Model file for the job. Use its own axes, mm. Face numbers are marked on the shaded views. A direction names the side the tool comes from. Round coordinates to 2 decimals unless told otherwise and drop trailing zeros. Loops run counter-clockwise (first coordinate to the right, second up) from the corner with the lowest first, then second, coordinate; pieces in that order, holes last. Notation, with made-up numbers: (-39.75, 33.5) - (11.25, 33.5) arc R21 cw to (11.25, 70.5) - close; hole circle Ø5 at (-10, 42.5). An arc over 180 degrees is marked (long way). Answer as a JSON object with one key per item and string values.
from build123d import *

# Parameters (mm, degrees)
SKETCH_1_R          = 37.5
EXTRUDE_1_DEPTH     = 12.5
FILLET_1_R          = 7
SKETCH_2_R          = 5.411787985
EXTRUDE_2_DEPTH     = 15
EXTRUDE_3_DEPTH     = 5
SKETCH_4_W          = 95
SKETCH_4_H          = 64
EXTRUDE_4_DEPTH     = 3
SKETCH_6_R          = 4.25
CUT_EXTRUDE_1_DEPTH = 141.349563667
SKETCH_9_W          = 92.539395388
SKETCH_9_H          = 8.982437317
CUT_EXTRUDE_2_DEPTH = 121.43878113
SKETCH_10_W         = 82.805159643
SKETCH_10_H         = 35
EXTRUDE_5_DEPTH     = 5
SKETCH_11_R         = 17.5
EXTRUDE_6_DEPTH     = 3.982437317
EXTRUDE_1_2_DEPTH   = 30


with BuildPart() as part:
    # Sketch 1 → Extrude 1 (new, symmetric)
    with BuildSketch(Plane.XY):
        Circle(SKETCH_1_R)
    extrude(amount=EXTRUDE_1_DEPTH, both=True)

    # Fillet 1
    fillet_1_edges = [part.edges().sort_by_distance(p)[0] for p in [
        (-37.5, 0, -12.5),
        (-37.5, 0, 12.5),
    ]]
    fillet(fillet_1_edges, radius=FILLET_1_R)

    # Sketch 2 → Extrude 2 (add, symmetric)
    with BuildSketch(Plane.XY):
        Circle(SKETCH_2_R)
    extrude(amount=EXTRUDE_2_DEPTH, both=True)

    # Sketch 3 → Extrude 3 (add)
    with BuildSketch(Plane.XY.offset(12.5)):
        with BuildLine():
            Line((-7.008676366, -7.132913542), (-85, 69.5))
            Line((-85, 69.5), (10, 69.5))
            Line((10, 69.5), (10, 0))
            ThreePointArc((10, 0), (3.867378721, -9.221896867), (-7.008676366, -7.132913542))
        make_face()
    extrude_3 = extrude(amount=EXTRUDE_3_DEPTH)

    # Mirror 1: Extrude 3 across plane
    add(extrude_3.mirror(Plane.XY))

    # Sketch 4 → Extrude 4 (add)
    with BuildSketch(Plane(origin=(0, 69.5, 0), x_dir=(1, 0, 0), z_dir=(0, 1, 0))):
        with Locations((-37.5, 0)):
            Rectangle(SKETCH_4_W, SKETCH_4_H)
    extrude(amount=-EXTRUDE_4_DEPTH)

    # Sketch 6 → Cut-Extrude 1 (cut, through all)
    with BuildSketch(Plane(origin=(0, 69.5, 0), x_dir=(1, 0, 0), z_dir=(0, 1, 0))):
        with Locations(Location((-0.5, -22.4, 0), (0, 0, 270))):
            Circle(SKETCH_6_R)
        with Locations(Location((-0.5, 22.4, 0), (0, 0, 270))):
            Circle(SKETCH_6_R)
        with Locations(Location((-74.5, 22.4, 0), (0, 0, 270))):
            Circle(SKETCH_6_R)
        with Locations(Location((-74.5, -22.4, 0), (0, 0, 270))):
            Circle(SKETCH_6_R)
    extrude(amount=-CUT_EXTRUDE_1_DEPTH, mode=Mode.SUBTRACT)

    # Sketch 9 → Cut-Extrude 2 (cut, through all)
    with BuildSketch(Plane.XY.offset(17.5)):
        with Locations((-36.269697694, 62.008781341)):
            Rectangle(SKETCH_9_W, SKETCH_9_H)
    extrude(amount=-CUT_EXTRUDE_2_DEPTH, mode=Mode.SUBTRACT)


with BuildPart() as cut_extrude_2_piece_1:
    # of the separate pieces the step leaves, piece 1, a body of its own (cut_extrude_2_pieces)
    add(part.part.solids().sort_by_distance((37.5, 0, -5.5))[0])

    # Sketch 10 → Extrude 5 (add)
    with BuildSketch(Plane(origin=(0, 57.517562683, 0), x_dir=(1, 0, 0), z_dir=(0, 1, 0))):
        with Locations((-31.402579822, 0)):
            Rectangle(SKETCH_10_W, SKETCH_10_H)
    extrude(amount=EXTRUDE_5_DEPTH)



with BuildPart() as cut_extrude_2_piece_2:
    # of the separate pieces the step leaves, piece 2, a body of its own (cut_extrude_2_pieces)
    add(part.part.solids().sort_by_distance((10, 66.5, 32))[0])


with BuildPart() as cut_extrude_2_piece_1_1:
    add(cut_extrude_2_piece_1.part)

    add(cut_extrude_2_piece_2.part)  # Extrude 6 merges Cut-Extrude 2 piece 2
    # Sketch 11 → Extrude 6 (add)
    with BuildSketch(Plane(origin=(0, 62.517562683, 0), x_dir=(1, 0, 0), z_dir=(0, 1, 0))):
        with Locations(Location((-31.402579821, 0, 0), (0, 0, 270))):
            Circle(SKETCH_11_R)
    extrude(amount=EXTRUDE_6_DEPTH)

    # Sketch 8 → Extrude 1 2 (add)
    with BuildSketch(Plane.XY.offset(17.5)):
        Polygon((-19.25, 45.79201997), (9.430275915, 45.79201997), (29.164495175, 28.274139716), (53.347206554, 28.274139716), (53.347206554, 31.274139716), (30.303943346, 31.274139716), (10.569724085, 48.79201997), (-19.25, 48.79201997), align=None)
    extrude(amount=-EXTRUDE_1_2_DEPTH)


solid = cut_extrude_2_piece_1_1.part
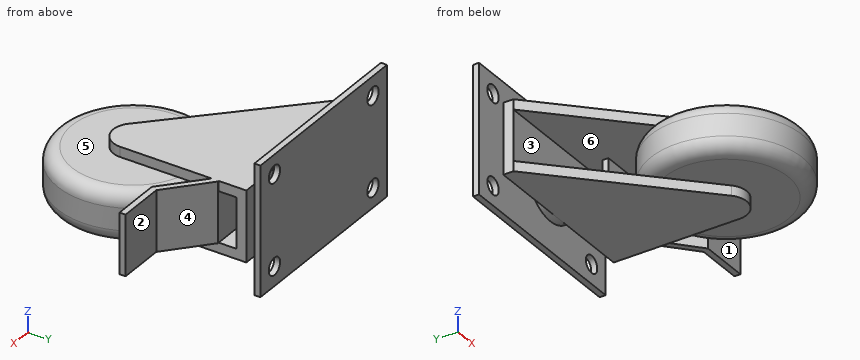
1) Tool access for the marked faces 1, 2 and 3: list every direction of +Z, -Z, +X, -X, +Y, -Y with a clear straight run to the whole face (end or side of a thin tool).
Values follow:
{"face 1": "+Z, -Z, +X", "face 2": "+Z, -Z, +X, +Y", "face 3": "+X, -X"}
2) Slice it at D-D on z = -2. List the corners of the cut face in (x, y).
Values follow:
{"outline": "(-85, 66.5) - (-48.79, 66.5) - (-48.79, 62.52) - (-72.81, 62.52) - (-72.81, 57.52) - (10, 57.52) - (10, 62.52) - (-14.02, 62.52) - (-14.02, 66.5) - (10, 66.5) - (10, 69.5) - (-85, 69.5) - close; circle Ø75 at (0, 0); (-19.25, 45.79) - (9.43, 45.79) - (29.16, 28.27) - (53.35, 28.27) - (53.35, 31.27) - (30.3, 31.27) - (10.57, 48.79) - (-19.25, 48.79) - close"}
3) Probe probe 1 along Z at (x, y) = (0, 68); probe 2 along X at (y, z) = (67.2, -22.4); probe 3 along Y at (x, z) = (-50.5, 6). List the from-to ranges inside material, lowest first.
Values follow:
{"probe 1": "-32 to -26.62, -18.18 to 18.18, 26.62 to 32", "probe 2": "-85 to -78.75, -70.25 to -4.75, 3.75 to 10", "probe 3": "57.52 to 62.52, 66.5 to 69.5"}
4) Slice it at C-C on x = -74.5. List the corners of the cut face in (y, z), then the cut area to 3 significant figures.
Values follow:
{"outline": "(66.5, -32) - (69.5, -32) - (69.5, -26.65) - (66.5, -26.65) - close; (66.5, -18.15) - (69.5, -18.15) - (69.5, 18.15) - (66.5, 18.15) - close; (66.5, 26.65) - (69.5, 26.65) - (69.5, 32) - (66.5, 32) - close", "area": "141 mm²"}
5) Drop flat-ended pins along their axis: P1, Ø12, axis at x = -15.5, z = 13, coming from the -Y side; P2, Ø1, axis at y = 23.5, z = 0.5, coming from the +X side; P3, Ø22, axis at x = -34.5, y = 38, coming from the +Z side. Give the stop position or say it passes through.
Values follow:
{"P1": "y = -34.99", "P2": "x = 29.62", "P3": "z = 17.5"}
6) Two-plate mould, pull along Y, no slides. Class the marked faces 4, 5 and 6: pulls with the +Y half, pulls with the -Y half, needs draft (parallel to the pull), parting line crosses it, or undercut.
Values follow:
{"face 4": "pulls with the +Y half", "face 5": "needs draft", "face 6": "undercut"}
7) Slice it at B-B on x = -56.5. List the corners of the cut face in (y, z), then the cut area to 3 significant figures.
Values follow:
{"outline": "(41.5, -17.5) - (62.52, -17.5) - (62.52, 17.5) - (41.5, 17.5) - (41.5, 12.5) - (57.52, 12.5) - (57.52, -12.5) - (41.5, -12.5) - close; (66.5, -32) - (69.5, -32) - (69.5, 32) - (66.5, 32) - close", "area": "527 mm²"}
8) Slice it at A-A on z = 22.4. List the corners of the cut face in (x, y).
Values follow:
{"outline": "(-85, 66.5) - (-78.75, 66.5) - (-78.75, 69.5) - (-85, 69.5) - close; (-70.25, 66.5) - (-4.75, 66.5) - (-4.75, 69.5) - (-70.25, 69.5) - close; (3.75, 66.5) - (10, 66.5) - (10, 69.5) - (3.75, 69.5) - close"}
